```python
from build123d import *

# Parameters (mm, degrees)
FRAME_PLATE_12MM_DEPTH      = 6
RIM_BOSS_DEPTH              = 10
FACE_RECESS_2MM_DEPTH       = 2
UPPER_START                 = 2
UPPER_RELIEF_CUT_SKETCH_R   = 25
UPPER_RELIEF_CUT_2MM_DEPTH  = 2
CENTRE_RELIEF_CUT_2MM_DEPTH = 2
LOWER_RELIEF_CUT_SKETCH_R   = 52.651518039
LOWER_RELIEF_CUT_2MM_DEPTH  = 2
JAW_OPENING_SKETCH_R        = 15
JAW_OPENING_CUT_DEPTH       = 125.85191228


with BuildPart() as part:
    # Frame Profile Sketch → Frame Plate 12mm (new, symmetric)
    with BuildSketch(Plane.XY):
        with BuildLine():
            Line((57.219040426, -50), (57.219040426, -38))
            Line((57.219040426, -38), (47.219040426, -38))
            Line((47.219040426, -38), (47.219040426, -50))
            ThreePointArc((47.219040426, -50), (43.953561552, -61.533330749), (35.126520593, -69.642857143))
            ThreePointArc((35.126520593, -69.642857143), (-77.659797107, 7.277081367), (47.453139554, 61.904761905))
            ThreePointArc((47.453139554, 61.904761905), (51.779005163, 56.637617931), (53.327535793, 50))
            Line((53.327535793, 50), (53.327535793, 38))
            Line((53.327535793, 38), (63.327535793, 38))
            Line((63.327535793, 38), (63.327535793, 50))
            ThreePointArc((63.327535793, 50), (60.74665141, 61.062696552), (53.536875394, 69.841269841))
            ThreePointArc((53.536875394, 69.841269841), (-87.616181352, 8.210040517), (39.629920669, -78.571428571))
            ThreePointArc((39.629920669, -78.571428571), (52.469252974, -66.775753816), (57.219040426, -50))
        make_face()
    extrude(amount=FRAME_PLATE_12MM_DEPTH, both=True)

    # Rim Boss Sketch → Rim Boss (add)
    with BuildSketch(Plane.XY.offset(6)):
        with BuildLine():
            Line((53.327535793, 38), (32.46615526, 38))
            ThreePointArc((32.46615526, 38), (13.979168764, 40.044097465), (15.696546582, 21.523902608))
            ThreePointArc((15.696546582, 21.523902608), (32.534616457, -2.315840538), (15.696546582, -26.155583684))
            ThreePointArc((15.696546582, -26.155583684), (12.648035491, -48.265354025), (32.46615526, -38))
            Line((32.46615526, -38), (47.219040426, -38))
            Line((47.219040426, -38), (47.219040426, -50))
            ThreePointArc((47.219040426, -50), (43.953561552, -61.533330749), (35.126520593, -69.642857143))
            ThreePointArc((35.126520593, -69.642857143), (-77.659797107, 7.277081367), (47.453139554, 61.904761905))
            ThreePointArc((47.453139554, 61.904761905), (51.779005163, 56.637617931), (53.327535793, 50))
            Line((53.327535793, 50), (53.327535793, 38))
        make_face()
    extrude(amount=-RIM_BOSS_DEPTH)

    # Face Recess Sketch → Face Recess 2mm (cut)
    with BuildSketch(Plane.XY.offset(6)):
        with BuildLine():
            ThreePointArc((36.866729899, -68.73750233), (44.45885626, -60.703554629), (47.219040426, -50))
            Line((47.219040426, -50), (47.219040426, -38))
            Line((47.219040426, -38), (32.46615526, -38))
            ThreePointArc((32.46615526, -38), (30.153940112, -45.264433679), (24.06810264, -49.855829743))
            ThreePointArc((24.06810264, -49.855829743), (7.879587743, -42.091412935), (15.644004551, -25.902898038))
            ThreePointArc((15.644004551, -25.902898038), (32.325529371, -3.417209672), (17.682148152, 20.445959399))
            ThreePointArc((17.682148152, 20.445959399), (16.663921846, 20.938096482), (15.696546582, 21.523902608))
            ThreePointArc((15.696546582, 21.523902608), (13.979168764, 40.044097465), (32.46615526, 38))
            Line((32.46615526, 38), (53.327535793, 38))
            Line((53.327535793, 38), (53.327535793, 50))
            ThreePointArc((53.327535793, 50), (51.779005163, 56.637617931), (47.453139554, 61.904761905))
            ThreePointArc((47.453139554, 61.904761905), (-77.745163176, 6.299968474), (36.866729899, -68.73750233))
        make_face()
    extrude(amount=-FACE_RECESS_2MM_DEPTH, mode=Mode.SUBTRACT)

    # Upper Relief Cut Sketch → Upper Relief Cut 2mm (cut)
    with BuildSketch(Plane.XY.offset(4).offset(UPPER_START)):
        with Locations((7.349665755, -2.318921614)):
            Circle(UPPER_RELIEF_CUT_SKETCH_R)
    extrude(amount=-UPPER_RELIEF_CUT_2MM_DEPTH, mode=Mode.SUBTRACT)

    # Centre Relief Cut Sketch → Centre Relief Cut 2mm (cut)
    with BuildSketch(Plane.XY.offset(4)):
        with BuildLine():
            ThreePointArc((23.833190109, -22.398989717), (-15.184880461, 28.968173855), (4.862308851, -32.34337094))
            ThreePointArc((4.862308851, -32.34337094), (27.276572021, -52.035475846), (23.833190109, -22.398989717))
        make_face()
    extrude(amount=CENTRE_RELIEF_CUT_2MM_DEPTH, mode=Mode.SUBTRACT)

    # Lower Relief Cut Sketch → Lower Relief Cut 2mm (cut)
    with BuildSketch(Plane.XY.offset(4)):
        with Locations((-7.330378767, 0)):
            Circle(LOWER_RELIEF_CUT_SKETCH_R)
    extrude(amount=LOWER_RELIEF_CUT_2MM_DEPTH, mode=Mode.SUBTRACT)

    # Jaw Opening Sketch → Jaw Opening Cut (cut, through all)
    with BuildSketch(Plane.XY.offset(4)):
        with Locations((-30.10151943, 0)):
            Circle(JAW_OPENING_SKETCH_R)
    extrude(amount=-JAW_OPENING_CUT_DEPTH, mode=Mode.SUBTRACT)


solid = part.part
```
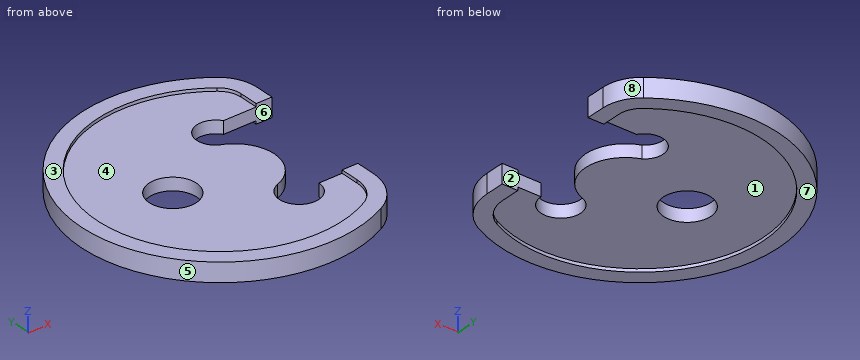
Verification items for the finished model (mm, model axes). Face numbers are marked on the shaded views. A direction names the side the tool comes from. Coordinates: 2 decimals unless noted, no trailing zeros. Write each loop counter-clockwise with the first axis right and the second up, starting at its lowest first coordinate (ties: lowest second). Pieces come first, ordered by that corner, then holes. Notation, with made-up numbers: M -13,-33 L 10,-33 A10 cw 10,-24 Z; hole C 12.25,-12.75 d3. An arc over 180 degrees is marked long. Answer as a JSON object with one key per item and string values. Group by question number.
(1) Cross-section at D-D, the plane y = 67.5. Record the cut outline in (x, z).
(2) Gauge pin test, flat ends, axial feed: pin 1 (2 mm diameter, centred on x = -45.5, y = 52.5, fed in from -Z); pin 2 (0.6 mm diameter, centred on y = -43.5, z = -5, fed in from -X); pin 3 (1 mm diameter, centred on y = 42.5, z = -5, fed in from -X); pin 4 (12 mm diameter, centred on x = 19.5, y = 29.5, fed in from +Z). Record the tip position at first contact, or that the pin passes through.
(3) Material ranges on line 1 (Y direction, x = 18, z = -3); line 2 (Y direction, x = 0, z = 5); line 3 (Z direction, x = -32.5, y = -41), recorded low to high.
(4) Cross-section at A-A, the plane z = -1.5. Record the cut outline in (x, y), and give its area (3 significant figures).
(5) Tool access check on the marked faces 1, 2, 3 and 4. Record the directions out of +Z, -Z, +X, -X, +Y, -Y that give a thin tool (end or side, any length) a straight path to the whole face; none if there is none.
(6) Cross-section at B-B, the plane x = 12.5. Record the cut outline in (y, z), and give its area (3 significant figures).
(7) Cross-section at C-C, the plane y = 0. Record the cut outline in (x, z).
(8) Release check for a two-part mould opening along Y. For the marked faces 5, 6, 7 and 8 record: +Y half, -Y half, draft (parallel to the pull), parting line (faces both ways), or undercut.
Reply:
{
 "1": {"outline": "M -56.46,-6 L -39.09,-6 L -39.09,-4 L 39.09,-4 L 39.09,-6 L 56.18,-6 L 56.18,6 L 39.09,6 L 39.09,4 L -39.09,4 L -39.09,6 L -56.46,6 Z"},
 "2": {"pin 1": "z = -4", "pin 2": "x = -76.67", "pin 3": "x = -77.33", "pin 4": "through"},
 "3": {"line 1": "-86.14 to -50.42, -25.21 to 20.58, 42.65 to 86.14", "line 2": "-88 to -78, 78 to 88", "line 3": "-4 to 4"},
 "4": {"outline": "M 15.7,-26.16 A25.3 ccw 15.7,21.52 A12 cw long 32.47,38 L 63.33,38 L 63.33,50 A25 ccw 53.54,69.84 A88 ccw long 39.63,-78.57 A32 ccw 57.22,-50 L 57.22,-38 L 32.47,-38 A12.57 cw long Z; hole C -30.1,0 d30", "area": "17,800 mm²"},
 "5": {"face 1": "-Z", "face 2": "+Z, -Z, +X", "face 3": "+Z, +X, -X, +Y, -Y", "face 4": "+Z"},
 "6": {"outline": "M -87.11,-6 L -76.99,-6 L -76.99,-4 L -48.16,-4 L -48.16,4 L -76.99,4 L -76.99,6 L -87.11,6 Z; M -27.84,-4 L 24.69,-4 L 24.69,4 L -27.84,4 Z; M 38.28,-4 L 76.99,-4 L 76.99,-6 L 87.11,-6 L 87.11,6 L 76.99,6 L 76.99,4 L 38.28,4 Z", "area": "1,200 mm²"},
 "7": {"outline": "M -88,-6 L -78,-6 L -78,-4 L -45.1,-4 L -45.1,4 L -78,4 L -78,6 L -88,6 Z; M -15.1,-4 L 32.43,-4 L 32.43,4 L -15.1,4 Z"},
 "8": {"face 5": "parting line", "face 6": "undercut", "face 7": "draft", "face 8": "+Y half"}
}
